```python
from build123d import *

# Parameters (mm, degrees)
SKETCH1_W           = 30
SKETCH1_H           = 40
BOSS_EXTRUDE1_DEPTH = 8
SKETCH2_W           = 30
SKETCH2_H           = 34
BOSS_EXTRUDE2_DEPTH = 8
SKETCH3_W           = 8
SKETCH3_H           = 15
BOSS_EXTRUDE3_DEPTH = 40
CHAMFER1_SIZE       = 5
BOSS_EXTRUDE4_DEPTH = 8
CHAMFER2_SIZE       = 20


with BuildPart() as part:
    # Sketch1 → Boss-Extrude1 (new body)
    with BuildSketch(Plane(origin=(0, 0, 0), x_dir=(1, 0, 0), z_dir=(0, 1, 0))):
        Rectangle(SKETCH1_W, SKETCH1_H)
    extrude(amount=BOSS_EXTRUDE1_DEPTH)

    # Sketch2 → Boss-Extrude2 (add)
    with BuildSketch(Plane.XY.offset(20)):
        with Locations((0, -9)):
            Rectangle(SKETCH2_W, SKETCH2_H)
    extrude(amount=BOSS_EXTRUDE2_DEPTH)

    # Sketch3 → Boss-Extrude3 (add)
    with BuildSketch(Plane.ZY.offset(15)):
        with Locations((24, -18.5)):
            Rectangle(SKETCH3_W, SKETCH3_H)
    extrude(amount=BOSS_EXTRUDE3_DEPTH)

    # Chamfer1
    chamfer1_edges = [part.edges().sort_by_distance(p)[0] for p in [
        (-55, -11, 24),
    ]]
    chamfer(chamfer1_edges, length=CHAMFER1_SIZE)

    # Sketch4 → Boss-Extrude4 (add)
    with BuildSketch(Plane(origin=(0, 0, 20), x_dir=(-1, 0, 0), z_dir=(0, 0, -1))):
        Polygon((30, -11), (50, -11), (55, -16), (55, -26), (30, -26), align=None)
    extrude(amount=BOSS_EXTRUDE4_DEPTH)

    # Chamfer2
    chamfer2_edges = [part.edges().sort_by_distance(p)[0] for p in [
        (15, -26, 24),
    ]]
    chamfer(chamfer2_edges, length=CHAMFER2_SIZE)


solid = part.part
```
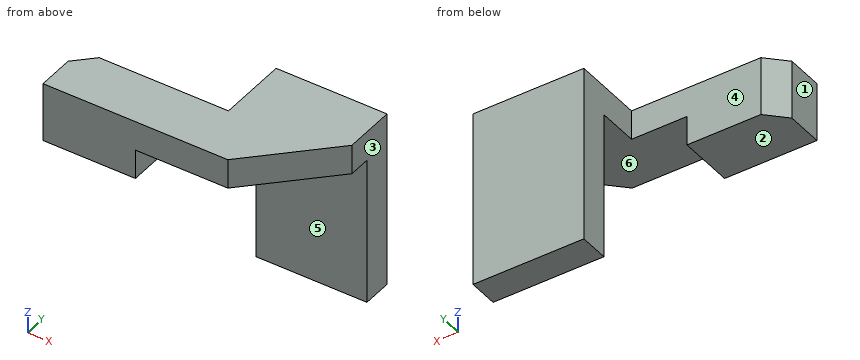
CAD build for the part. Positions are in the model's coordinates, mm. Face numbers are marked on the shaded views. A direction names the side the tool comes from. Give positions to 0.01 mm unless a question says otherwise; leave off trailing zeros. Loops run counter-clockwise (first coordinate to the right, second up) from the corner with the lowest first, then second, coordinate; pieces in that order, holes last. Notation, with made-up numbers: M -16.75,-27 L -10.75,-27 A17 cw -10.75,-4 Z; hole C -1.75,0 d11. An arc over 180 degrees is marked long. Use one line per item in the form item = value.
Item 1: Drill centre lines: probe 1 along Y at (x, z) = (-12.5, -1.5); probe 2 along Z at (x, y) = (-4.5, -4.5); probe 3 along X at (y, z) = (5, 5). Where is each one in solid material? Low to high. Write a range as from..to.
Determined:
probe_1 = 0..8
probe_2 = 20..28
probe_3 = -15..15
Item 2: Slice it at A-A (z = 18). List the corners of the cut face in (x, y).
Determined:
outline = M -55,-26 L -30,-26 L -30,-11 L -50,-11 L -55,-16 Z; M -15,0 L 15,0 L 15,8 L -15,8 Z
Item 3: Slice it at D-D (z = 10). List the corners of the cut face in (x, y), plus the area to 3 significant figures.
Determined:
outline = M -15,0 L 15,0 L 15,8 L -15,8 Z
area = 240 mm2
Item 4: Which spindle directions (+Z, -Z, +X, -X, +Y, -Y) get a long thin tool onto all of the face, cutting with end or side? Do the marked faces 4, 5 and 6. Say none if no direction does.
Determined:
face_4 = +Z, -Z, -X, +Y
face_5 = -Z, +X, -X, -Y
face_6 = -Z, +X, -Y
Item 5: Slice it at C-C (y = -9). List the corners of the cut face in (x, z), plus the area to 3 significant figures.
Determined:
outline = M -15,20 L 12,20 L 12,28 L -15,28 Z
area = 216 mm2
Item 6: Two-plate mould, pull along X, no slides. Class the marked faces 1, 2 and 3: pulls with the +X half, pulls with the -X half, needs draft (parallel to the pull), parting line crosses it, or undercut.
Determined:
face_1 = pulls with the -X half
face_2 = needs draft
face_3 = pulls with the +X half
Item 7: Slice it at B-B (x = 10). List the corners of the cut face in (y, z), plus the area to 3 significant figures.
Determined:
outline = M -11,20 L 0,20 L 0,-20 L 8,-20 L 8,28 L -11,28 Z
area = 472 mm2
Item 8: Flat gauge pins, fed straight in: pin 1 (5.5 mm diameter, centred on y = 3, z = 7.5, fed in from -X); pin 2 (2.5 mm diameter, centred on y = -18.5, z = 16, fed in from +X); pin 3 (8 mm diameter, centred on x = -35.5, z = 24, fed in from +Y). Where does each tip first touch, or does it go through?
Determined:
pin_1 = -15
pin_2 = -30
pin_3 = -11
